```python
from build123d import *

# Parameters (mm, degrees)
BASE_BLOCK_SKETCH_W       = 89
BASE_BLOCK_SKETCH_H       = 40
BASE_BLOCK_50MM_DEPTH     = 50
ROUNDED_BOSS_44MM_DEPTH   = 44
BOSS_START                = 44
BOSS_EXTENSION_44MM_DEPTH = 44
GUSSET_A_16MM_DEPTH       = 16
RECESS_START              = -4
RECESS_4MM_DEPTH          = 4
PAD_START                 = 4
PAD_4MM_DEPTH             = 4
GUSSET_B_16MM_DEPTH       = 16
BORE_SKETCH_50_R          = 25
BORE_50_DEPTH             = 88
SIDE_SLOT_DEPTH           = 50
HOLE_SKETCH_12_R          = 6
HOLE_12_DEPTH             = 10


with BuildPart() as part:
    # Base Block Sketch → Base Block 50mm (new body)
    with BuildSketch(Plane.XY):
        with Locations((44.5, -20)):
            Rectangle(BASE_BLOCK_SKETCH_W, BASE_BLOCK_SKETCH_H)
    extrude(amount=BASE_BLOCK_50MM_DEPTH)

    # Rounded Boss Sketch → Rounded Boss 44mm (add)
    with BuildSketch(Plane(origin=(0, 0, 0), x_dir=(1, 0, 0), z_dir=(0, 1, 0))):
        with BuildLine():
            Line((89, 0), (89, -16))
            Line((89, -16), (89, -50))
            ThreePointArc((89, -50), (126.5, -87.5), (164, -50))
            Line((164, -50), (164, -16))
            Line((164, -16), (164, 0))
            Line((164, 0), (89, 0))
        make_face()
    extrude(amount=-ROUNDED_BOSS_44MM_DEPTH)

    # Boss Extension Sketch → Boss Extension 44mm (add)
    with BuildSketch(Plane(origin=(0, 0, 0), x_dir=(1, 0, 0), z_dir=(0, 1, 0)).offset(BOSS_START)):
        with BuildLine():
            Line((164, 0), (164, -50))
            ThreePointArc((164, -50), (126.5, -87.5), (89, -50))
            Line((89, -50), (89, 0))
            Line((89, 0), (164, 0))
        make_face()
    extrude(amount=-BOSS_EXTENSION_44MM_DEPTH)

    # Gusset A Sketch → Gusset A 16mm (add)
    with BuildSketch(Plane(origin=(0, 0, 0), x_dir=(-1, 0, 0), z_dir=(0, 0, -1))):
        Polygon((-89, 44), (-89, 0), (0, 0), align=None)
    extrude(amount=-GUSSET_A_16MM_DEPTH)

    # Recess Sketch → Recess 4mm (cut)
    with BuildSketch(Plane.XZ.offset(44).offset(RECESS_START)):
        with BuildLine():
            Line((89, 0), (89, 50))
            ThreePointArc((89, 50), (126.5, 87.5), (164, 50))
            Line((164, 50), (164, 0))
            Line((164, 0), (89, 0))
        make_face()
    extrude(amount=RECESS_4MM_DEPTH, mode=Mode.SUBTRACT)

    # Pad Sketch → Pad 4mm (add)
    with BuildSketch(Plane(origin=(0, 44, 0), x_dir=(1, 0, 0), z_dir=(0, 1, 0)).offset(PAD_START)):
        with BuildLine():
            Line((89, 0), (164, 0))
            Line((164, 0), (164, -50))
            ThreePointArc((164, -50), (126.5, -87.5), (89, -50))
            Line((89, -50), (89, 0))
        make_face()
    extrude(amount=-PAD_4MM_DEPTH)

    # Gusset B Sketch → Gusset B 16mm (add)
    with BuildSketch(Plane(origin=(0, 0, 0), x_dir=(-1, 0, 0), z_dir=(0, 0, -1))):
        Polygon((-89, 48), (-89, 44), (0, 0), align=None)
    extrude(amount=-GUSSET_B_16MM_DEPTH)

    # Bore Sketch Ø50 → Bore Ø50 (cut)
    with BuildSketch(Plane(origin=(0, 48, 0), x_dir=(1, 0, 0), z_dir=(0, 1, 0))):
        with Locations(Location((126.5, -50, 0), (0, 0, 270))):
            Circle(BORE_SKETCH_50_R)
    extrude(amount=-BORE_50_DEPTH, mode=Mode.SUBTRACT)

    # Side Slot Sketch → Side Slot (cut)
    with BuildSketch(Plane.XY.offset(50)):
        with BuildLine():
            Line((25.5, -29), (63.5, -29))
            ThreePointArc((63.5, -29), (74.5, -18), (63.5, -7))
            Line((63.5, -7), (25.5, -7))
            ThreePointArc((25.5, -7), (14.5, -18), (25.5, -29))
        make_face()
    extrude(amount=-SIDE_SLOT_DEPTH, mode=Mode.SUBTRACT)

    # Hole Sketch Ø12 → Hole Ø12 (cut)
    with BuildSketch(Plane(origin=(0, 0, 0), x_dir=(1, 0, 0), z_dir=(0, 1, 0))):
        with Locations(Location((44, -33, 0), (0, 0, 270))):
            Circle(HOLE_SKETCH_12_R)
    extrude(amount=-HOLE_12_DEPTH, mode=Mode.SUBTRACT)


solid = part.part
```
Design review of the part built by this model. Coordinates are the model's own, in mm. A direction names the side the tool comes from. Coordinates: 2 decimals unless noted, no trailing zeros. Order: outer loops, then holes, each group sorted by start corner. A loop starts at its lowest first (then second) coordinate and runs counter-clockwise, first axis right, second up.
1) Take a section at D-D, the plane x = 44. Give the boundary of the cut face in (y, z), and give its area (3 significant figures).
2) Wall thickness on line 1 along Y through (x, z) = (43, 42); line 2 along Z through (x, y) = (126, 8) (3 decimals); line 3 along X through (y, z) = (22, 50): over which ranges is each line inside the solid? List them lowest first.
3) For faces 5 (the cylindrical face through (44, -3, 27)), 6 (the flat face through (164, 5, 25)), 7 (the flat face through (65, 14, 16)), 8 (the flat face through (44, -33, 50)), 9 (the flat face through (44, -29, 25)), list the 3-axis set-ups (+Z, -Z, +X, -X, +Y, -Y) from which the entire face can be reached by the end or side of a thin tool; tool diameter is ignored.
4) Take a section at B-B, the plane y = -18. Give the boundary of the cut face in (x, z).
5) Take a section at C-C, the plane z = 12.5. Give the boundary of the cut face in (x, y), and give its area (3 significant figures).
6) Clearance check with flat-ended pins moving along their axes: pin 1 (12 mm diameter, centred on x = 25.5, z = 47.5, fed in from +Y); pin 2 (17 mm diameter, centred on y = 32, z = 35, fed in from -X); pin 3 (1 mm diameter, centred on y = 13, z = 16, fed in from -X). State where each tip first meets the part, or that it passes through.
7) Take a section at A-A, the plane x = 126.5. Give the boundary of the cut face in (y, z), and give its area (3 significant figures).
8) Mouldability with a two-part tool opening along Y and no side actions: class faces 1 (the flat face through (45, -7, 25)), 2 (the cylindrical face through (127.32, 4.62, 87.49)), 3 (the cylindrical face through (74.5, -18.2, 25.4)), 4 (the flat face through (81, -40, 33)) as +Y half, -Y half, draft (parallel to the pull), parting line (faces both ways), or undercut.
Returned:
1. outline: (-40, 0) - (-29, 0) - (-29, 50) - (-40, 50) - close; (-7, 0) - (23.73, 0) - (23.73, 16) - (0, 16) - (0, 27) - (-7, 27) - close; (-7, 39) - (0, 39) - (0, 50) - (-7, 50) - close
1. area: 1,200 mm2
2. line 1: y = -40 to -29, -7 to 0
2. line 2: z = 0 to 25.005, 74.995 to 87.497
2. line 3: x = 89 to 101.5, 151.5 to 164
3. face 5: +Y
3. face 6: +Z, -Z, +X, +Y, -Y
3. face 7: +Z, -X, +Y
3. face 8: +Z, -X, +Y, -Y
3. face 9: +Z, -Z
4. outline: (0, 0) - (14.5, 0) - (14.5, 50) - (0, 50) - close; (74.5, 0) - (164, 0) - (164, 50) arc R37.5 ccw to (89, 50) - (74.5, 50) - close; hole circle Ø50 at (126.5, 50)
5. outline: (0, -40) - (164, -40) - (164, 48) - (89, 48) - (0, 0) - close; hole (25.5, -29) - (63.5, -29) arc R11 ccw to (63.5, -7) - (25.5, -7) arc R11 ccw to start
5. area: 11,100 mm2
6. pin 1: stops at y = 0
6. pin 2: stops at x = 89
6. pin 3: stops at x = 23.18
7. outline: (-40, 0) - (48, 0) - (48, 25) - (-40, 25) - close; (-40, 75) - (48, 75) - (48, 87.5) - (-40, 87.5) - close
7. area: 3,300 mm2
8. face 1: undercut
8. face 2: draft
8. face 3: undercut
8. face 4: -Y half
